The model under review builds one solid part; all positions refer to its coordinate system, in mm. A direction names the side the tool comes from. Give positions to 0.01 mm unless a question says otherwise; leave off trailing zeros. Order: outer loops, then holes, each group sorted by start corner. A loop starts at its lowest first (then second) coordinate and runs counter-clockwise, first axis right, second up. Notation, with made-up numbers: (-15.5, 35) - (41.5, 35) arc R11 ccw to (41.5, 45) - close; hole circle Ø6 at (34.25, -39). An arc over 180 degrees is marked (long way). Use CSV: the item, a comma, the result in double quotes.
```python
from build123d import *

# Parameters (mm, degrees)
BOSS_EXTRUDE1_DEPTH = 50
SKETCH2_R           = 24
BOSS_EXTRUDE2_DEPTH = 43
SKETCH3_R           = 38
BOSS_EXTRUDE3_DEPTH = 30
BOSS_EXTRUDE4_START = 477
SKETCH4_R           = 24
BOSS_EXTRUDE4_DEPTH = 477
CHAMFER1_SIZE       = 2


with BuildPart() as part:
    # Sketch1 → Boss-Extrude1 (new body)
    with BuildSketch(Plane.XY):
        Polygon((20.784609691, 12), (0, 24), (-20.784609691, 12), (-20.784609691, -12), (0, -24), (20.784609691, -12), align=None)
    extrude(amount=BOSS_EXTRUDE1_DEPTH)

    # Sketch2 → Boss-Extrude2 (add)
    with BuildSketch(Plane.XY.offset(50)):
        with Locations(Location((0, 0, 0), (0, 0, 150))):
            Circle(SKETCH2_R)
    extrude(amount=BOSS_EXTRUDE2_DEPTH)

    # Sketch3 → Boss-Extrude3 (add)
    with BuildSketch(Plane.XY.offset(93)):
        Circle(SKETCH3_R)
    extrude(amount=BOSS_EXTRUDE3_DEPTH)

    # Sketch4 → Boss-Extrude4 (add)
    with BuildSketch(Plane(origin=(0, 0, 0), x_dir=(-1, 0, 0), z_dir=(0, 0, -1)).offset(BOSS_EXTRUDE4_START)):
        with Locations(Location((0, 0, 0), (0, 0, 30))):
            Circle(SKETCH4_R)
    extrude(amount=-BOSS_EXTRUDE4_DEPTH)

    # Chamfer1
    chamfer1_edges = [part.edges().sort_by_distance(p)[0] for p in [
        (-38, 0, 93),
        (-38, 0, 123),
        (20.784609691, -12, -477),
    ]]
    chamfer(chamfer1_edges, length=CHAMFER1_SIZE)


solid = part.part
```
Item 1: Mouldability with a two-part tool opening along Z and no side actions: class faces 1 (the face through (20.785, 0, 25)), 2 (the face through (7.5, -23.5, 93)), 3 (the face through (-1, 1, 123)) as pulls with the +Z half, pulls with the -Z half, needs draft (parallel to the pull), parting line crosses it, or undercut.
Results list:
face 1,"undercut"
face 2,"pulls with the -Z half"
face 3,"pulls with the +Z half"
Item 2: Take a section at A-A, the plane y = 0. Give the boundary of the cut face in (x, z).
Results list:
outline,"(-38, 95) - (-36, 93) - (-24, 93) - (-24, 50) - (-20.78, 50) - (-20.78, 0) - (-24, 0) - (-24, -475) - (-22, -477) - (22, -477) - (24, -475) - (24, 0) - (20.78, 0) - (20.78, 50) - (24, 50) - (24, 93) - (36, 93) - (38, 95) - (38, 121) - (36, 123) - (-36, 123) - (-38, 121) - close"
Item 3: Wall thickness on L1, parallel to Z at x = 34.5, y = 2; L2, parallel to X at y = -12, z = 21; L3, parallel to Y at x = 8, z = -118.5: over which ranges is each line inside the solid? List them lowest first.
Results list:
L1,"z = 93 to 123"
L2,"x = -20.78 to 20.78"
L3,"y = -22.63 to 22.63"
Item 4: Tool access review of faces 4 (the face through (-11, 19, 0)), 5 (the face through (11, 19, 50)), 6 (the face through (-7.21, -22.89, -240.82)), 7 (the face through (10.25, -18.08, 24.65)), 8 (the face through (-20.785, 0, 25)): name each direction out of +Z, -Z, +X, -X, +Y, -Y from which nothing blocks a thin tool from reaching the whole face with its end or side.
Results list:
face 4,"-X, +Y"
face 5,"+X, +Y"
face 6,"-Z"
face 7,"+X, -Y"
face 8,"-X, +Y, -Y"
Item 5: Clearance check with flat-ended pins moving along their axes: pin 1 (12 mm diameter, centred on y = -22, z = -234.5, fed in from +X); pin 2 (1 mm diameter, centred on x = 7, y = -25, fed in from -Z); pin 3 (4 mm diameter, centred on x = 13.5, z = -121, fed in from +Y); pin 4 (4 mm diameter, centred on x = -26.5, z = -376.5, fed in from +Y). State where each tip first meets the part, or that it passes through.
Results list:
pin 1,"stops at x = 17.89"
pin 2,"stops at z = 93"
pin 3,"stops at y = 21.07"
pin 4,"passes through"
Item 6: Take a section at B-B, the plane z = -255.5. Give the boundary of the cut face in (x, y).
Results list:
outline,"circle Ø48 at (0, 0)"
